CAD build for the part. Positions are in the model's coordinates, mm. Coordinates: 2 decimals unless noted, no trailing zeros. Order: outer loops, then holes, each group sorted by start corner. A loop starts at its lowest first (then second) coordinate and runs counter-clockwise, first axis right, second up. Notation, with made-up numbers: (-5.5, -37) - (2.5, -37) arc R25 cw to (2.5, -6) - close; hole circle Ø10 at (35.5, 26.25). An arc over 180 degrees is marked (long way). Write each question's results on one line, items separated by ' | '. Start each with the question number.
Q1. Band-saw the part on C-C, the plane x = -24. Write the cut outline in (y, z).
Q2. Band-saw the part on A-A, the plane x = -50. Write the cut outline in (y, z).
Q3. Pull direction X, two halves, no side cores. Call faces 1 (the cylindrical face through (45.954, -34.822, -0.021)), 2 (the flat face through (-1, -55, 0)), 3 (the cylindrical face through (-52.985, 37.737, -0.021)), 4 (the flat face through (-70, -1, 0)): released by +X, released by -X, zero draft, split by the parting line, or undercut.
Q4. Band-saw the part on B-B, the plane y = 47. Write the cut outline in (x, z).
Q5. Wall check: probe 1 along Y at (x, z) = (62, -0.1); probe 2 along Y at (x, z) = (-50, 0); probe 3 along X at (y, z) = (-46, -0.3). Give the ranges that are in metal, low to high.
Q6. Band-saw the part on D-D, the plane y = 35. Write the cut outline in (x, z), then the cut area to 3 significant figures.
```python
from build123d import *

# Parameters (mm, degrees)
SKETCH_1_W      = 140
SKETCH_1_H      = 110
SKETCH_1_R      = 2.25
SKETCH_1_R_2    = 4.05
EXTRUDE_1_DEPTH = 1.5


with BuildPart() as part:
    # 草图1 → 凸台-拉伸1 (new, symmetric)
    with BuildSketch(Plane.XY):
        Rectangle(SKETCH_1_W, SKETCH_1_H)
        with Locations((-62, -47)):
            Circle(SKETCH_1_R, mode=Mode.SUBTRACT)
        with Locations((-62, 47)):
            Circle(SKETCH_1_R, mode=Mode.SUBTRACT)
        with Locations((62, -47)):
            Circle(SKETCH_1_R, mode=Mode.SUBTRACT)
        with Locations((62, 47)):
            Circle(SKETCH_1_R, mode=Mode.SUBTRACT)
        with Locations((-50, -35)):
            Circle(SKETCH_1_R_2, mode=Mode.SUBTRACT)
        with Locations((-50, 35)):
            Circle(SKETCH_1_R_2, mode=Mode.SUBTRACT)
        with Locations((50, -35)):
            Circle(SKETCH_1_R_2, mode=Mode.SUBTRACT)
        with Locations((50, 35)):
            Circle(SKETCH_1_R_2, mode=Mode.SUBTRACT)
        with Locations((-24, 35)):
            Circle(SKETCH_1_R, mode=Mode.SUBTRACT)
    extrude(amount=EXTRUDE_1_DEPTH, both=True)


solid = part.part
```
Results below:
1) outline: (-55, -1.5) - (32.75, -1.5) - (32.75, 1.5) - (-55, 1.5) - close; (37.25, -1.5) - (55, -1.5) - (55, 1.5) - (37.25, 1.5) - close
2) outline: (-55, -1.5) - (-39.05, -1.5) - (-39.05, 1.5) - (-55, 1.5) - close; (-30.95, -1.5) - (30.95, -1.5) - (30.95, 1.5) - (-30.95, 1.5) - close; (39.05, -1.5) - (55, -1.5) - (55, 1.5) - (39.05, 1.5) - close
3) face 1: undercut | face 2: zero draft | face 3: undercut | face 4: released by -X
4) outline: (-70, -1.5) - (-64.25, -1.5) - (-64.25, 1.5) - (-70, 1.5) - close; (-59.75, -1.5) - (59.75, -1.5) - (59.75, 1.5) - (-59.75, 1.5) - close; (64.25, -1.5) - (70, -1.5) - (70, 1.5) - (64.25, 1.5) - close
5) probe 1: y = -55 to -49.25, -44.75 to 44.75, 49.25 to 55 | probe 2: y = -55 to -39.05, -30.95 to 30.95, 39.05 to 55 | probe 3: x = -70 to -64.02, -59.98 to 59.98, 64.02 to 70
6) outline: (-70, -1.5) - (-54.05, -1.5) - (-54.05, 1.5) - (-70, 1.5) - close; (-45.95, -1.5) - (-26.25, -1.5) - (-26.25, 1.5) - (-45.95, 1.5) - close; (-21.75, -1.5) - (45.95, -1.5) - (45.95, 1.5) - (-21.75, 1.5) - close; (54.05, -1.5) - (70, -1.5) - (70, 1.5) - (54.05, 1.5) - close | area: 358 mm²
